CAD build for the part. Positions are in the model's coordinates, mm. A direction names the side the tool comes from. Coordinates: 2 decimals unless noted, no trailing zeros. Order: outer loops, then holes, each group sorted by start corner. A loop starts at its lowest first (then second) coordinate and runs counter-clockwise, first axis right, second up. Notation, with made-up numbers: M 57,36 L 80,36 A9 ccw 80,43 Z; hole C -26,56.25 d10. An arc over 180 degrees is marked long. One line per item, written item: value.
from build123d import *

# Parameters (mm, degrees)
SKETCH1_W           = 1002
SKETCH1_H           = 1427
BOSS_EXTRUDE1_DEPTH = 2
CUT_EXTRUDE1_DEPTH  = 2
BOSS_EXTRUDE2_DEPTH = 30


with BuildPart() as part:
    # Sketch1 → Boss-Extrude1 (new body)
    with BuildSketch(Plane.XY):
        Rectangle(SKETCH1_W, SKETCH1_H)
    extrude(amount=BOSS_EXTRUDE1_DEPTH)

    # Sketch2 → Cut-Extrude1 (cut)
    with BuildSketch(Plane.XY.offset(2)):
        Polygon((-419.25, 713.5), (501, -713.5), (501, 713.5), align=None)
    extrude(amount=-CUT_EXTRUDE1_DEPTH, mode=Mode.SUBTRACT)

    # Sketch4 → Boss-Extrude2 (add)
    with BuildSketch(Plane(origin=(0, 0, 0), x_dir=(-1, 0, 0), z_dir=(0, 0, -1))):
        Polygon((420.340042889, 711.5), (-497.33041962, -711.5), (499, -711.5), (499, 711.5), (501, 713.5), (501, -713.5), (-501, -713.5), (419.25, 713.5), align=None)
    extrude(amount=BOSS_EXTRUDE2_DEPTH)


solid = part.part
Q1. Slice it at A-A (z = -23). List the corners of the cut face in (x, y).
Recorded:
outline: M -501,-713.5 L 501,-713.5 L -419.25,713.5 L -420.34,711.5 L 497.33,-711.5 L -499,-711.5 L -499,711.5 L -501,713.5 Z
Q2. Which spindle directions (+Z, -Z, +X, -X, +Y, -Y) get a long thin tool onto all of the face, cutting with end or side? Do faces 1 (the face through (47.317, -9.989, -13.776)), 2 (the face through (-499, -10, -15)), 3 (the face through (-120, -147, 0)). Say none if no direction does.
Recorded:
face 1: +Z, -Z, +X, +Y
face 2: -Z, +Y
face 3: -Z
Q3. Slice it at B-B (y = 173). List the corners of the cut face in (x, z), plus the area to 3 significant figures.
Recorded:
outline: M -501,-30 L -499,-30 L -499,0 L -73.07,0 L -73.07,-30 L -70.69,-30 L -70.69,2 L -501,2 Z
area: 992 mm^2
Q4. Pin check, flat tips, straight feed: pin 1 Ø6 at (x, z) = (-241.5, -17.5) entering from +Y; pin 2 Ø3 at (y, z) = (-510, -13.5) entering from +X; pin 3 Ø9 at (y, z) = (57.5, -14.5) entering from +X. Stop position of each tip, or through.
Recorded:
pin 1: stops at y = 442.52
pin 2: stops at x = 370.73
pin 3: stops at x = 6.7
Q5. Drill centre lines: line 1 along X through (y, z) = (-29, -12.5); line 2 along X through (y, z) = (-16.5, -18.5); line 3 along Y through (x, z) = (215, -24). Where is each one in solid material? Low to high.
Recorded:
line 1: x = -501 to -499, 57.2 to 59.58
line 2: x = -501 to -499, 49.14 to 51.52
line 3: y = -713.5 to -711.5, -273.7 to -270.01
Q6. Mould opens along X. For faces 4 (the face through (-501, 10, -14)), 5 (the face through (6, -711.5, -15)), 6 (the face through (-118, -149, 2)) say: released by +X, released by -X, zero draft, split by the parting line, or undercut.
Recorded:
face 4: released by -X
face 5: undercut
face 6: zero draft
